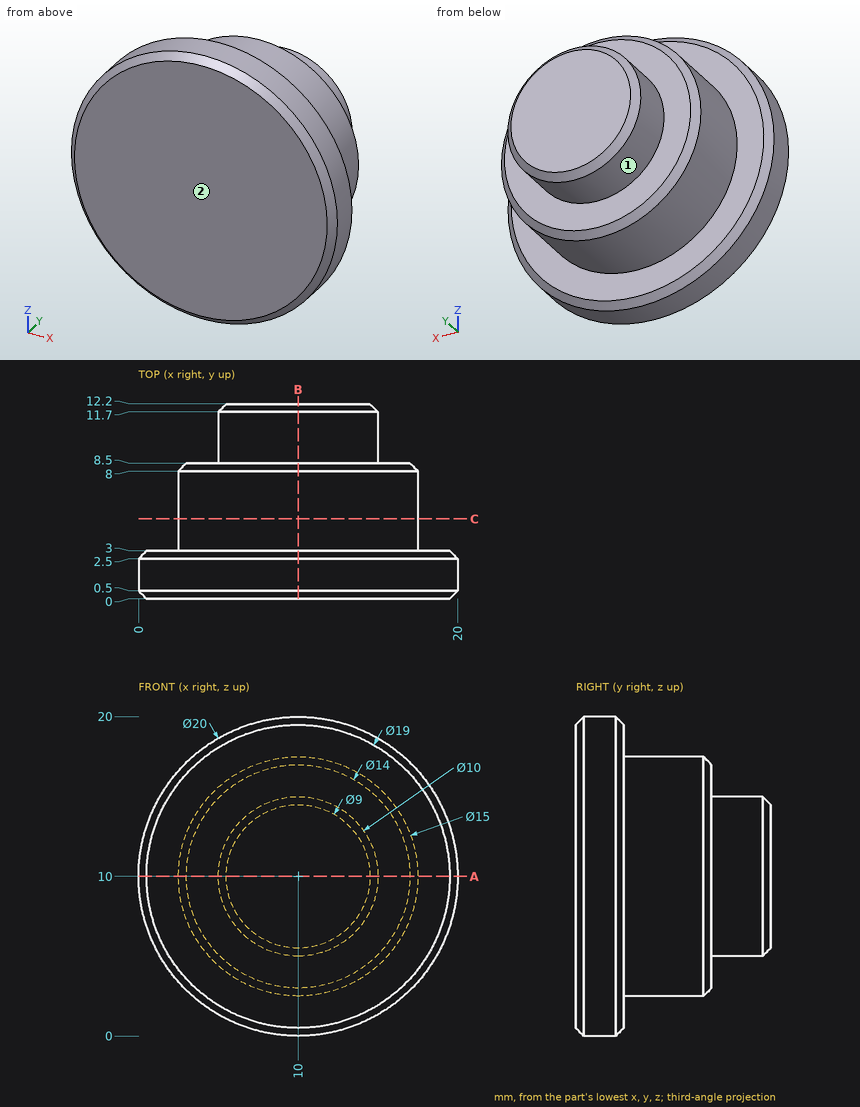
Study the drawing (mm; zero at the part's minimum x, y, z) and answer. A direction names the side the tool comes from. Coordinates: 2 decimals unless noted, no trailing zeros. Loops run counter-clockwise (first coordinate to the right, second up) from the corner with the lowest first, then second, coordinate; pieces in that order, holes last. Notation, with made-up numbers: (10, 69) -> (25, 69) arc R28 ccw to (25, 99) -> close; hole circle Ø2 at (6, 40.5). An arc over 180 degrees is marked (long way). Answer in a Markdown table with one row per item. Add a question column.
1. Flat-ended cylindrical pins translate along their axes: P1, Ø3, axis at x = 16, y = 3.5, coming from the -Z side; P2, Ø2, axis at x = 4.5, y = 10, coming from the +Z side; P3, Ø5, axis at x = 11, y = 6, coming from the +Z side. Find the tip coordinate at first contact, or state that the pin passes through.
2. The part is cut by section A-A, the plane z = 10. Write down the section's boundary in (x, y).
3. The part is cut by section C-C, the plane y = 5. Write down the section's boundary in (x, z), then the cut area to 3 significant figures.
4. Consider line 1 (Y direction, x = 4.5, z = 2.75); line 2 (Y direction, x = 11, z = 16); line 3 (Z direction, x = 13.75, y = 2). Determine where each line is inside the solid, lowest interval first. Write a range as [from, to].
5. The part is cut by section B-B, the plane x = 10. Write down the section's boundary in (y, z), then the cut area to 4 significant figures.
6. For the marked faces 1 and 2, determine the directions among +Z, -Z, +X, -X, +Y, -Y from which every point of the face is accessible in a straight line to the end or side of a thin tool.
Answer below:
| question | item | result |
|---|---|---|
| 1 | P1 | z = 1.27 |
| 1 | P2 | z = 12.18 |
| 1 | P3 | z = 17.5 |
| 2 | outline | (0, 0.5) -> (0.5, 0) -> (19.5, 0) -> (20, 0.5) -> (20, 2.5) -> (19.5, 3) -> (17.5, 3) -> (17.5, 8) -> (17, 8.5) -> (15, 8.5) -> (15, 11.7) -> (14.5, 12.2) -> (5.5, 12.2) -> (5, 11.7) -> (5, 8.5) -> (3, 8.5) -> (2.5, 8) -> (2.5, 3) -> (0.5, 3) -> (0, 2.5) -> close |
| 3 | outline | circle Ø15 at (10, 10) |
| 3 | area | 177 mm2 |
| 4 | line 1 | [0, 3] |
| 4 | line 2 | [0, 8.5] |
| 4 | line 3 | [0.73, 19.27] |
| 5 | outline | (0, 0.5) -> (0.5, 0) -> (2.5, 0) -> (3, 0.5) -> (3, 2.5) -> (8, 2.5) -> (8.5, 3) -> (8.5, 5) -> (11.7, 5) -> (12.2, 5.5) -> (12.2, 14.5) -> (11.7, 15) -> (8.5, 15) -> (8.5, 17) -> (8, 17.5) -> (3, 17.5) -> (3, 19.5) -> (2.5, 20) -> (0.5, 20) -> (0, 19.5) -> close |
| 5 | area | 178.5 mm2 |
| 6 | face 1 | +Y |
| 6 | face 2 | +Z, -Z, +X, -X, -Y |
